Answer from the drawing. Dimensions are ordinates in mm from the lowest x, y and z of the part. Coordinates: 2 decimals unless noted, no trailing zeros. Order: outer loops, then holes, each group sorted by start corner. A loop starts at its lowest first (then second) coordinate and runs counter-clockwise, first axis right, second up. Notation, with made-up numbers: (43, 42) -> (67, 42) arc R25 ccw to (67, 68) -> close; hole circle Ø2 at (-1, -6.75). An arc over 180 degrees is marked (long way). Use CSV: the item, a comma, the result in double quotes.
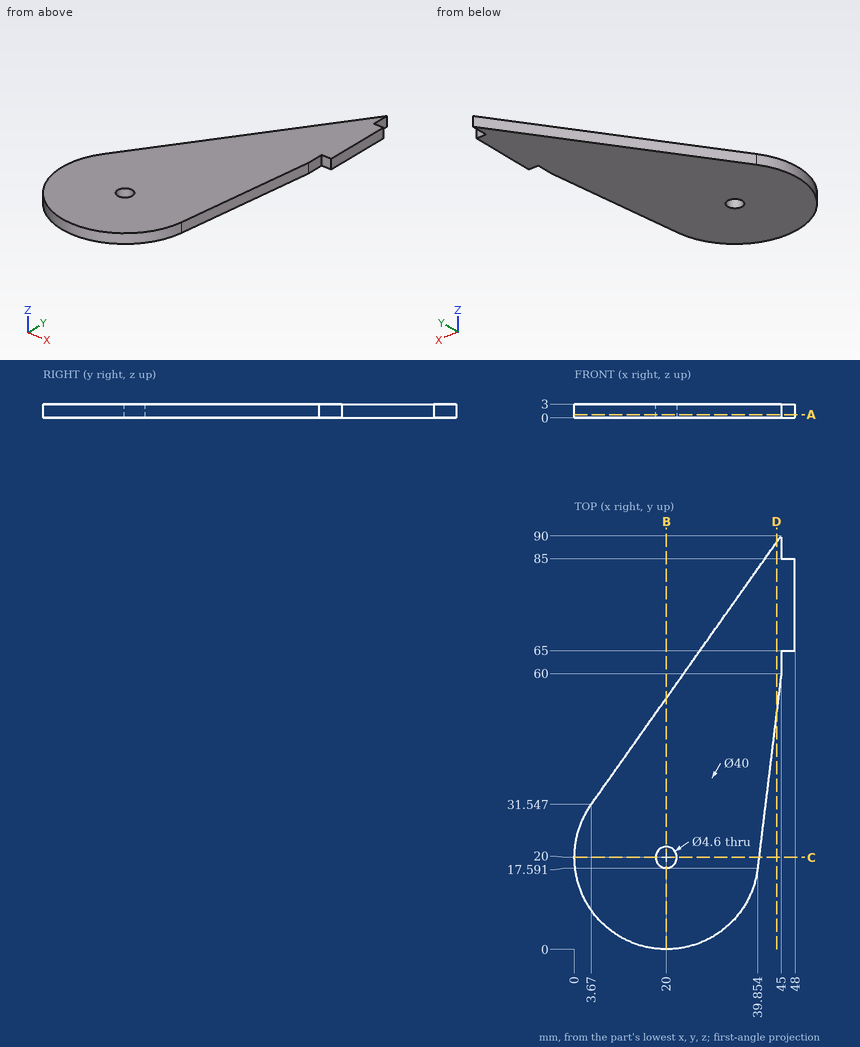
Item 1: Straight lines are drawn through the part: line 1 along Y through (x, z) = (20, 2.1) (1 decimal); line 2 along Y through (x, z) = (46.5, 2.35); line 3 along X through (y, z) = (86.5, 2.5) (1 decimal). For each, find the intervals that lie inside material, in ascending order.
Return value:
line 1,"y = 0 to 17.7, 22.3 to 54.6"
line 2,"y = 65 to 85"
line 3,"x = 42.5 to 45"
Item 2: Find section C-C, the plane y = 20. Give the vertices of the cut face in (x, z), then the cut area to 3 significant figures.
Return value:
outline,"(0, 0) -> (17.7, 0) -> (17.7, 3) -> (0, 3) -> close; (22.3, 0) -> (40.15, 0) -> (40.15, 3) -> (22.3, 3) -> close"
area,"107 mm^2"
Item 3: Find section D-D, the plane x = 44. Give the vertices of the cut face in (y, z) (1 decimal).
Return value:
outline,"(51.8, 0) -> (88.6, 0) -> (88.6, 3) -> (51.8, 3) -> close"
Item 4: Find section B-B, the plane x = 20. Give the vertices of the cut face in (y, z), then the cut area to 3 significant figures.
Return value:
outline,"(0, 0) -> (17.7, 0) -> (17.7, 3) -> (0, 3) -> close; (22.3, 0) -> (54.64, 0) -> (54.64, 3) -> (22.3, 3) -> close"
area,"150 mm^2"
Item 5: Each of these flat-tipped pins is pushed along its axis until it touches: P1, Ø1.5, axis at x = 46.5, z = 2, coming from the -Y side; P2, Ø0.9, axis at y = 87.5, z = 1, coming from the +X side; P3, Ø8, axis at x = 15, y = 57, coming from the -Z side; P4, Ø1, axis at x = 43, z = 1, coming from the +Y side. Where does it stop, or does it pass through?
Return value:
P1,"stops at y = 65"
P2,"stops at x = 45"
P3,"passes through"
P4,"stops at y = 87.88"
Item 6: Find section A-A, the plane z = 0.7. Give the vertices of the cut face in (x, y) (1 decimal), then the cut area to 3 significant figures.
Return value:
outline,"(3.7, 31.5) arc R20 ccw (long way) to (39.9, 17.6) -> (45, 60) -> (45, 65) -> (48, 65) -> (48, 85) -> (45, 85) -> (45, 90) -> close; hole circle Ø4.6 at (20, 20)"
area,"2,290 mm^2"
